from build123d import *

# Parameters (mm, degrees)
SKETCH2_R          = 3.5
CUT_EXTRUDE1_DEPTH = 10
FILLET1_R          = 3
SKETCH3_W          = 36
SKETCH3_H          = 90
CUT_EXTRUDE2_DEPTH = 151.332963784
CIRPATTERN1_COUNT  = 3
SKETCH4_W          = 114.578796514
SKETCH4_H          = 147.158368746
CUT_EXTRUDE3_DEPTH = 151.332963784


with BuildPart() as part:
    # Sketch1 → Revolve1 (revolve)
    with BuildSketch(Plane.XY, mode=Mode.PRIVATE) as revolve1_sk:
        Polygon((0, 40), (0, 68), (74, 68), (74, 90), (80, 90), (80, 58), (30, 58), (30, 50.919107028), align=None)
    revolve(revolve1_sk.sketch.rotate(Axis((0, 0, 0), (1, 0, 0)), 90), axis=Axis((0, 0, 0), (1, 0, 0)))

    # Sketch2 → Cut-Extrude1 (cut)
    with BuildSketch(Plane(origin=(80, 0, 0), x_dir=(0, 0, -1), z_dir=(1, 0, 0))):
        with Locations((0, 80)):
            Circle(SKETCH2_R)
        with Locations((69.282032303, 40)):
            Circle(SKETCH2_R)
        with Locations((69.282032303, -40)):
            Circle(SKETCH2_R)
        with Locations((0, -80)):
            Circle(SKETCH2_R)
        with Locations((-69.282032303, -40)):
            Circle(SKETCH2_R)
        with Locations((-69.282032303, 40)):
            Circle(SKETCH2_R)
    extrude(amount=-CUT_EXTRUDE1_DEPTH, mode=Mode.SUBTRACT)

    # Fillet1
    fillet1_edges = [part.edges().sort_by_distance(p)[0] for p in [
        (74, 0, -68),
    ]]
    fillet(fillet1_edges, radius=FILLET1_R)

    # Sketch3 → Cut-Extrude2 (cut, through all)
    with BuildSketch(Plane(origin=(0, 0, 0), x_dir=(1, 0, 0), z_dir=(0, 1, 0))):
        with Locations((51, 0)):
            Rectangle(SKETCH3_W, SKETCH3_H)
    cut_extrude2 = extrude(amount=-CUT_EXTRUDE2_DEPTH, mode=Mode.SUBTRACT)

    # CirPattern1: Cut-Extrude2 ×3 about axis
    cirpattern1_axis = Axis((0, 0, 0), (1, 0, 0))
    for i in range(1, CIRPATTERN1_COUNT):
        add(cut_extrude2.rotate(cirpattern1_axis, i * 360 / CIRPATTERN1_COUNT), mode=Mode.SUBTRACT)

    # Sketch4 → Cut-Extrude3 (cut, through all)
    with BuildSketch(Plane.ZY):
        with Locations((57.289398257, 73.579184373)):
            Rectangle(SKETCH4_W, SKETCH4_H)
    extrude(amount=-CUT_EXTRUDE3_DEPTH, mode=Mode.SUBTRACT)


solid = part.part
Model file for the job. Use its own axes, mm. A direction names the side the tool comes from. Give positions to 0.01 mm unless a question says otherwise; leave off trailing zeros. Loops run counter-clockwise (first coordinate to the right, second up) from the corner with the lowest first, then second, coordinate; pieces in that order, holes last.
1) Tool access for faces 4 (the flat face through (50.75, 60.81, -15.33)), 5 (the flat face through (31, 62, 0)), 6 (the flat face through (51, -44, -45)): list every direction of +Z, -Z, +X, -X, +Y, -Y with a clear straight run to the whole face (end or side of a thin tool).
2) Pull direction Y, two halves, no side cores. Call faces 1 (the flat face through (50.75, -17.13, -60.33)), 2 (the cylindrical face through (69.698, -47.874, -32.743)), 3 (the flat face through (51, -44, 45)): +Y half, -Y half, draft (parallel to the pull), parting line (faces both ways), or undercut.
3) Wall check: line 1 (X direction, y = 36.5, z = -63); line 2 (Z direction, x = 33.5, y = -19); line 3 (Y direction, x = 40, z = -0.5). Give the ranges that are in metal, low to high.
4) Saw through at C-C (z = -7). Count the separate pieces of the cut face and the enclosed holes in it, plus the area to 3 significant figures.
5) Saw through at B-B (y = -80). Write the cut outline in (x, z), plus the area to 3 significant figures.
6) Saw through at D-D (x = 14). Write the cut outline in (y, z).
7) Flat gauge pins, fed straight in: pin 1 Ø9 at (x, z) = (72.5, 75) entering from +Y; pin 2 Ø5.5 at (y, z) = (40, -69.28) entering from -X; pin 3 Ø11.5 at (x, y) = (54, -42) entering from -Z; pin 4 Ø4 at (x, y) = (51.5, -21.5) entering from +Z. Where does each tip first touch, or does it go through?
8) Saw through at A-A (x = 52.5). Write the cut outline in (y, z).
Answer block:
1. face 4: -Z, -Y
1. face 5: +Z, +X, -X, +Y
1. face 6: +Y, -Y
2. face 1: +Y half
2. face 2: undercut
2. face 3: draft
3. line 1: x = 74 to 80
3. line 2: z = -65.29 to -57.09, 57.09 to 65.29
3. line 3: y = 58 to 68
4. separate pieces: 3
4. enclosed holes: 0
4. area: 2,280 mm2
5. outline: (74, -41.23) - (80, -41.23) - (80, -3.5) - (74, -3.5) - close; (74, 3.5) - (80, 3.5) - (80, 41.23) - (74, 41.23) - close
5. area: 453 mm2
6. outline: (0, 45.1) - (0, 68) arc R68 ccw (long way) to (68, 0) - (45.1, 0) arc R45.1 cw (long way) to start
7. pin 1: stops at y = 0
7. pin 2: passes through
7. pin 3: stops at z = -57.53
7. pin 4: stops at z = 65.14
8. outline: (-50.98, -45) arc R68 ccw to (-13.48, -66.65) - (-20.67, -54.19) arc R58 cw to (-36.59, -45) - close; (-50.98, 45) - (-36.59, 45) arc R58 cw to (-20.67, 54.19) - (-13.48, 66.65) arc R68 ccw to start; (57.27, -9.19) - (64.46, -21.65) arc R68 ccw to (68, 0) - (58, 0) arc R58 cw to start
